Here's how the part is built. I have some questions about the finished solid (model axes, mm). A direction names the side the tool comes from. Round coordinates to 2 decimals unless told otherwise and drop trailing zeros. Order: outer loops, then holes, each group sorted by start corner. A loop starts at its lowest first (then second) coordinate and runs counter-clockwise, first axis right, second up. Notation, with made-up numbers: M -19.5,18 L 38.5,18 A21 cw 38.5,54 Z; hole C 88.5,52.25 d3. An arc over 180 degrees is marked long. Write item = value, one per line. Start each with the question number.
Item 1: I want a section at D-D, the plane y = 13.5. List the corners of the cut face in (x, z) for me.
Item 2: I'm going to push flat-ended pins straight in: P1, Ø10, axis at x = 34, z = -16.5, coming from the -Y side; P2, Ø12, axis at x = -34, z = -20.5, coming from the +Y side; P3, Ø5.5, axis at y = -3, z = -6, coming from the +X side. Where does each tip first touch, or does it pass through?
Item 3: I want a section at A-A, the plane y = 8.5. List the corners of the cut face in (x, z) for me.
Item 4: We'd pull the mould along X, two halves only. Please class faces 1 (the face through (5.681, 10.647, -0.466)), 2 (the face through (13, 21, 0)), 3 (the face through (-43, 19, 0)): pulls with the +X half, pulls with the -X half, needs draft (parallel to the pull), parting line crosses it, or undercut.
Item 5: I want a section at B-B, the plane z = -10. List the corners of the cut face in (x, y) for me, plus the area to 3 significant figures.
Item 6: Please list where these lines run through material, in increasing order: L1, parallel to Z at x = 3, y = 5.75; L2, parallel to Y at x = -21, z = -23; L3, parallel to X at y = 8.25, z = 6.
Item 7: For faces 4 (the face through (-28, 0, 0)), 5 (the face through (3, 0, 6)), 6 (the face through (11, 26, -26)), 7 (the face through (30, 0, 0)), 8 (the face through (31.42, 16.56, 17.8)), which set-ups out of +Z, -Z, +X, -X, +Y, -Y let a thin tool reach every point of the face, with its end or its side?
Item 8: I want a section at C-C, the plane x = -13.5. List the corners of the cut face in (y, z) for me, plus the area to 3 significant figures.
```python
from build123d import *

# Parameters (mm, degrees)
BASE_BLOCK_SKETCH_W         = 86
BASE_BLOCK_SKETCH_H         = 64
BASE_BLOCK_86X64X39_DEPTH   = 39
ANGLED_SIDE_CUT_25DEG_DEPTH = 129
TOP_STEP_CUT_SKETCH_R       = 7
TOP_STEP_CUT_DEPTH          = 18
CORNER_BEVEL_CUT_DEPTH      = 27
THROUGH_HOLE_SKETCH_R       = 7
THROUGH_HOLE_DEPTH          = 97
GUIDE_TONGUE_SKETCH_W       = 30
GUIDE_TONGUE_SKETCH_H       = 7
GUIDE_TONGUE_DEPTH          = 64


with BuildPart() as part:
    # Base Block Sketch → Base Block 86x64x39 (new body)
    with BuildSketch(Plane(origin=(0, 0, 0), x_dir=(1, 0, 0), z_dir=(0, 1, 0))):
        Rectangle(BASE_BLOCK_SKETCH_W, BASE_BLOCK_SKETCH_H)
    extrude(amount=BASE_BLOCK_86X64X39_DEPTH)

    # Angled Side Cut Sketch → Angled Side Cut 25deg (cut)
    with BuildSketch(Plane(origin=(43, 0, 0), x_dir=(0, 0, -1), z_dir=(1, 0, 0))):
        Polygon((8, 39), (32, 27.808616204), (32, 39), align=None)
    extrude(amount=-ANGLED_SIDE_CUT_25DEG_DEPTH, mode=Mode.SUBTRACT)

    # Top Step Cut Sketch → Top Step Cut (cut)
    with BuildSketch(Plane(origin=(0, 39, 0), x_dir=(1, 0, 0), z_dir=(0, 1, 0))):
        Polygon((11, 32), (11, 20), (-32.633180821, -32), (19.502668792, -32), (43, -3.996971117), (43, 32), align=None)
        with Locations(Location((3, -6, 0), (0, 0, 270))):
            Circle(TOP_STEP_CUT_SKETCH_R, mode=Mode.SUBTRACT)
    extrude(amount=-TOP_STEP_CUT_DEPTH, mode=Mode.SUBTRACT)

    # Corner Bevel Cut Sketch → Corner Bevel Cut (cut)
    with BuildSketch(Plane(origin=(0, 39, 0), x_dir=(1, 0, 0), z_dir=(0, 1, 0))):
        Polygon((43, -3.996971117), (19.502668792, -32), (43, -32), align=None)
    extrude(amount=-CORNER_BEVEL_CUT_DEPTH, mode=Mode.SUBTRACT)

    # Through Hole Sketch → Through Hole (cut)
    with BuildSketch(Plane(origin=(0, 39, 0), x_dir=(1, 0, 0), z_dir=(0, 1, 0))):
        with Locations(Location((3, -6, 0), (0, 0, 90))):
            Circle(THROUGH_HOLE_SKETCH_R)
    extrude(amount=-THROUGH_HOLE_DEPTH, mode=Mode.SUBTRACT)

    # Guide Tongue Sketch → Guide Tongue (add)
    with BuildSketch(Plane.XY.offset(32)):
        with Locations((3, -3.5)):
            Rectangle(GUIDE_TONGUE_SKETCH_W, GUIDE_TONGUE_SKETCH_H)
    extrude(amount=-GUIDE_TONGUE_DEPTH)


solid = part.part
```
Filled in:
q1.outline = M -43,-32 L 43,-32 L 43,4 L 19.5,32 L -43,32 Z; hole C 3,6 d14
q2.P1 = 0
q2.P2 = 35.97
q2.P3 = 18
q3.outline = M -43,-32 L 43,-32 L 43,32 L -43,32 Z; hole C 3,6 d14
q4.face_1 = undercut
q4.face_2 = needs draft
q4.face_3 = pulls with the -X half
q5.outline = M -43,0 L -12,0 L -12,-7 L 18,-7 L 18,0 L 43,0 L 43,21 L 2.61,21 L 2.61,38.07 L -43,38.07 Z
q5.area = 2,790 mm^2
q6.L1 = -32 to -1, 13 to 32
q6.L2 = 0 to 32.01
q6.L3 = -43 to -4, 10 to 43
q7.face_4 = +Z, -Z, -X, -Y
q7.face_5 = +Y
q7.face_6 = +Z, -Z, +X, +Y
q7.face_7 = +Z, -Z, +X, -Y
q7.face_8 = +Z, +X, +Y
q8.outline = M 0,-32 L 27.81,-32 L 39,-8 L 39,9.2 L 21,9.2 L 21,32 L 0,32 Z
q8.area = 1,950 mm^2
